from build123d import *

# Parameters (mm, degrees)
SKETCH1_W                                            = 58
SKETCH1_H                                            = 32
BOSS_EXTRUDE1_DEPTH                                  = 10
CBORE_FOR_M4_HEXAGON_SOCKET_HEAD_CAP_SCR_D           = 3.4
CBORE_FOR_M4_HEXAGON_SOCKET_HEAD_CAP_SCR_DEPTH       = 18.1
CBORE_FOR_M4_HEXAGON_SOCKET_HEAD_CAP_SCR_CBORE_D     = 6
CBORE_FOR_M4_HEXAGON_SOCKET_HEAD_CAP_SCR_CBORE_DEPTH = 3.4
CBORE_FOR_M4_HEXAGON_SOCKET_HEAD_CAP_SCR_TIP         = 1.021463052
M6_TAPPED_HOLE1_D                                    = 5
M6_TAPPED_HOLE1_DEPTH                                = 15
M6_TAPPED_HOLE1_TIP                                  = 1.502151548
M8_TAPPED_HOLE1_D                                    = 6.8
M8_TAPPED_HOLE1_DEPTH                                = 19.75
M8_TAPPED_HOLE1_TIP                                  = 2.042926105
CHAMFER1_SIZE                                        = 3


with BuildPart() as part:
    # Sketch1 → Boss-Extrude1 (new body)
    with BuildSketch(Plane(origin=(0, 0, 0), x_dir=(1, 0, 0), z_dir=(0, 1, 0))):
        Rectangle(SKETCH1_W, SKETCH1_H)
    extrude(amount=BOSS_EXTRUDE1_DEPTH)

    # CBORE for M4 Hexagon socket head cap screws1
    with Locations(Plane(origin=(0, 0, 0), x_dir=(-1, 0, 0), z_dir=(0, -1, 0))):
        with Locations((-15, 12.5), (5, 12.5), (-15, -12.5), (5, -12.5)):
            CounterBoreHole(CBORE_FOR_M4_HEXAGON_SOCKET_HEAD_CAP_SCR_D / 2, CBORE_FOR_M4_HEXAGON_SOCKET_HEAD_CAP_SCR_CBORE_D / 2, CBORE_FOR_M4_HEXAGON_SOCKET_HEAD_CAP_SCR_CBORE_DEPTH, depth=CBORE_FOR_M4_HEXAGON_SOCKET_HEAD_CAP_SCR_DEPTH)
            with Locations((0, 0, -(CBORE_FOR_M4_HEXAGON_SOCKET_HEAD_CAP_SCR_DEPTH + CBORE_FOR_M4_HEXAGON_SOCKET_HEAD_CAP_SCR_TIP / 2))):  # 118° drill point
                Cone(0, CBORE_FOR_M4_HEXAGON_SOCKET_HEAD_CAP_SCR_D / 2, CBORE_FOR_M4_HEXAGON_SOCKET_HEAD_CAP_SCR_TIP, mode=Mode.SUBTRACT)

    # M6 Tapped Hole1
    with Locations(Plane(origin=(0, 0, 0), x_dir=(-1, 0, 0), z_dir=(0, -1, 0))):
        with Locations((19, 10), (19, -10)):
            Hole(M6_TAPPED_HOLE1_D / 2, depth=M6_TAPPED_HOLE1_DEPTH)
            with Locations((0, 0, -(M6_TAPPED_HOLE1_DEPTH + M6_TAPPED_HOLE1_TIP / 2))):  # 118° drill point
                Cone(0, M6_TAPPED_HOLE1_D / 2, M6_TAPPED_HOLE1_TIP, mode=Mode.SUBTRACT)

    # M8 Tapped Hole1
    with Locations(Plane(origin=(0, 0, 0), x_dir=(-1, 0, 0), z_dir=(0, -1, 0))):
        with Locations((-19, 0)):
            Hole(M8_TAPPED_HOLE1_D / 2, depth=M8_TAPPED_HOLE1_DEPTH)
            with Locations((0, 0, -(M8_TAPPED_HOLE1_DEPTH + M8_TAPPED_HOLE1_TIP / 2))):  # 118° drill point
                Cone(0, M8_TAPPED_HOLE1_D / 2, M8_TAPPED_HOLE1_TIP, mode=Mode.SUBTRACT)

    # Chamfer1
    chamfer1_edges = [part.edges().sort_by_distance(p)[0] for p in [
        (29, 5, 16),
        (-29, 5, 16),
        (-29, 5, -16),
        (29, 5, -16),
    ]]
    chamfer(chamfer1_edges, length=CHAMFER1_SIZE)


solid = part.part
Source: CAD feature listing. Evaluate the final solid. Frame: model axes, mm. A direction names the side the tool comes from. Round coordinates to 2 decimals unless told otherwise and drop trailing zeros. Order: outer loops, then holes, each group sorted by start corner. A loop starts at its lowest first (then second) coordinate and runs counter-clockwise, first axis right, second up. Notation, with made-up numbers: (84.25, 36) -> (93.25, 36) arc R21 ccw to (93.25, 65) -> close; hole circle Ø7 at (64.25, 31). An arc over 180 degrees is marked (long way). Answer as CSV lines item,"result".
Item 1: Pull-direction query (X, two-part tool) for faces 3 (the face through (16.57, 6.75, -11.85)), 4 (the face through (0, 10, 0)), 5 (the face through (28, 5, -14)); classes: pulls with the +X half, pulls with the -X half, needs draft (parallel to the pull), parting line crosses it, or undercut.
A:
face 3,"undercut"
face 4,"needs draft"
face 5,"pulls with the +X half"
Item 2: Line query: L1, parallel to Z at x = 15, y = 8; L2, parallel to Z at x = 15, y = 1.15; L3, parallel to X at y = 4.75, z = 13. Output: solid intervals per line, ascending.
A:
L1,"-16 to -14.2, -10.8 to 10.8, 14.2 to 16"
L2,"-16 to -15.5, -9.5 to 9.5, 15.5 to 16"
L3,"-29 to -6.62, -3.38 to 13.38, 16.62 to 29"
Item 3: Section B-B, the plane y = 2.5. Return loops of the section in (x, z), plus the area to 3 significant figures.
A:
outline,"(-29, -13) -> (-26, -16) -> (26, -16) -> (29, -13) -> (29, 13) -> (26, 16) -> (-26, 16) -> (-29, 13) -> close; hole circle Ø5 at (-19, -10); hole circle Ø5 at (-19, 10); hole circle Ø6 at (-5, -12.5); hole circle Ø6 at (-5, 12.5); hole circle Ø6 at (15, -12.5); hole circle Ø6 at (15, 12.5); hole circle Ø6.8 at (19, 0)"
area,"1,650 mm²"
Item 4: Pin query (flat end, axial travel): pin 1 Ø2.5 at (x, z) = (15, 12.5) entering from -Y; pin 2 Ø3 at (x, z) = (16, 13.5) entering from -Y; pin 3 Ø8 at (x, z) = (-5, -12.5) entering from +Y. Return the tip coordinate at first contact, or that it passes through.
A:
pin 1,"through"
pin 2,"y = 3.4"
pin 3,"y = 10"
Item 5: Section C-C, the plane x = 15. Return loops of the section in (y, z).
A:
outline,"(0, -16) -> (10, -16) -> (10, -14.2) -> (3.4, -14.2) -> (3.4, -15.5) -> (0, -15.5) -> close; (0, -9.5) -> (3.4, -9.5) -> (3.4, -10.8) -> (10, -10.8) -> (10, 10.8) -> (3.4, 10.8) -> (3.4, 9.5) -> (0, 9.5) -> close; (0, 15.5) -> (3.4, 15.5) -> (3.4, 14.2) -> (10, 14.2) -> (10, 16) -> (0, 16) -> close"
Item 6: Reachability of faces 1 (the face through (-4.086, 6.746, 11.067)), 2 (the face through (-5, 3.4, -10.5)) from +Z, -Z, +X, -X, +Y, -Y: full face, straight path, thin tool, end or side. Return the list, or none.
A:
face 1,"+Y, -Y"
face 2,"-Y"
Item 7: Section D-D, the plane z = -11.5. Return loops of the section in (x, y).
A:
outline,"(-29, 0) -> (-21, 0) -> (-21, 10) -> (-29, 10) -> close; (-17, 0) -> (-7.83, 0) -> (-7.83, 3.4) -> (-6.37, 3.4) -> (-6.37, 10) -> (-17, 10) -> close; (-3.63, 3.4) -> (-2.17, 3.4) -> (-2.17, 0) -> (12.17, 0) -> (12.17, 3.4) -> (13.63, 3.4) -> (13.63, 10) -> (-3.63, 10) -> close; (16.37, 3.4) -> (17.83, 3.4) -> (17.83, 0) -> (29, 0) -> (29, 10) -> (16.37, 10) -> close"
Item 8: Section A-A, the plane z = 0. Return loops of the section in (x, y).
A:
outline,"(-29, 0) -> (15.6, 0) -> (15.6, 10) -> (-29, 10) -> close; (22.4, 0) -> (29, 0) -> (29, 10) -> (22.4, 10) -> close"
